```python
from build123d import *
from build123d.topology import SkipClean

# Parameters (mm, degrees)
LUG_DEPTH                         = 19
LUG_PIN_HOLE_A_SKETCH_R           = 3
LUG_PIN_HOLE_A_6_DEPTH            = 19
LUG_PIN_HOLE_B_SKETCH_R           = 3
LUG_PIN_HOLE_B_6_DEPTH            = 19
LUG_PATTERN_3X120_COUNT           = 3
LUG_CHAMFER_4MM_SIZE              = 4
BORE_START                        = -3.5
BORE_RECESS_SKETCH_R              = 10
BORE_RECESS_20_X3_5_DEPTH         = 3.5
CENTRE_BORE_SKETCH_R              = 10
CENTRE_BORE_20_X7_DEPTH           = 7
COUNTERBORE_SKETCH_R              = 13
COUNTERBORE_26_X2_5_DEPTH         = 2.5
RADIAL_SLOT_PROFILE_R             = 4.75
RADIAL_SLOT_DEPTH                 = 5
FLANGE_HOLE_SKETCH_R              = 2.75
FLANGE_HOLE_5_5_DEPTH             = 50.979995998
SLOT_AND_HOLE_PATTERN_3X120_COUNT = 3


with BuildPart() as part:
    # Base Flange Profile → Base Flange Ø62 (revolve)
    with BuildSketch(Plane.XY):
        with BuildLine():
            Line((-31, 4), (-31, -4))
            Line((-31, -4), (-17, -4))
            Line((-17, -4), (-17, -7))
            Line((-17, -7), (-19, -7))
            ThreePointArc((-19, -7), (-19.707106781, -7.292893219), (-20, -8))
            Line((-20, -8), (-20, -9))
            Line((-20, -9), (0, -9))
            Line((0, -9), (0, 4))
            Line((0, 4), (-31, 4))
        make_face()
    revolve(axis=Axis((0, 39.539668131, 0), (0, -1, 0)))

    # Lug Profile → Lug (add)
    with SkipClean():  # the faces are left unmerged after this step: merging them gives an invalid solid
        with BuildSketch(Plane(origin=(0, 4, 0), x_dir=(1, 0, 0), z_dir=(0, 1, 0))):
            with BuildLine():
                Line((5, 30.594117082), (5, 8.660254038))
                ThreePointArc((5, 8.660254038), (8.660254038, 5), (10, 0))
                Line((10, 0), (28.995282599, -10.966931522))
                ThreePointArc((28.995282599, -10.966931522), (29.806622049, -8.518525814), (30.411611519, -6.011146713))
                Line((30.411611519, -6.011146713), (10, 5.773502692))
                Line((10, 5.773502692), (10, 29.342801502))
                ThreePointArc((10, 29.342801502), (7.526051267, 30.072554802), (5, 30.594117082))
            make_face()
        lug = extrude(amount=LUG_DEPTH)

    # Lug Pin Hole A Sketch → Lug Pin Hole A Ø6 (cut)
    with SkipClean():  # the faces are left unmerged after this step: merging them gives an invalid solid
        with BuildSketch(Plane.ZY.offset(-5)):
            with Locations((-25.594117082, 15)):
                Circle(LUG_PIN_HOLE_A_SKETCH_R)
        lug_pin_hole_a_6 = extrude(amount=-LUG_PIN_HOLE_A_6_DEPTH, mode=Mode.SUBTRACT)

    # Lug Pin Hole B Sketch → Lug Pin Hole B Ø6 (cut)
    with SkipClean():  # the faces are left unmerged after this step: merging them gives an invalid solid
        with BuildSketch(Plane(origin=(2.5, 0, -4.330127019), x_dir=(0.8660254037844399, 0, 0.4999999999999978), z_dir=(-0.4999999999999978, 0, 0.8660254037844399))):
            with Locations((25.594117082, 15)):
                Circle(LUG_PIN_HOLE_B_SKETCH_R)
        lug_pin_hole_b_6 = extrude(amount=-LUG_PIN_HOLE_B_6_DEPTH, mode=Mode.SUBTRACT)

    # Lug Pattern 3x120°: Lug, Lug Pin Hole A Ø6, Lug Pin Hole B Ø6 ×3 about axis
    with SkipClean():  # the faces are left unmerged after this step: merging them gives an invalid solid
        lug_pattern_3x120_axis = Axis((0, 0, 0), (0, 1, 0))
        add([lug.rotate(lug_pattern_3x120_axis, i * 360 / LUG_PATTERN_3X120_COUNT) for i in range(1, LUG_PATTERN_3X120_COUNT)])
        add([lug_pin_hole_a_6.rotate(lug_pattern_3x120_axis, i * 360 / LUG_PATTERN_3X120_COUNT) for i in range(1, LUG_PATTERN_3X120_COUNT)], mode=Mode.SUBTRACT)
        add([lug_pin_hole_b_6.rotate(lug_pattern_3x120_axis, i * 360 / LUG_PATTERN_3X120_COUNT) for i in range(1, LUG_PATTERN_3X120_COUNT)], mode=Mode.SUBTRACT)

    # Lug Chamfer 4mm
    lug_chamfer_4mm_edges = [part.edges().sort_by_distance(p)[0] for p in [
        (29.806622049, 23, 8.518525814),
        (7.526051267, 23, -30.072554802),
        (-7.526051267, 23, -30.072554802),
        (-29.806622049, 23, 8.518525814),
        (-22.280570782, 23, 21.554028988),
        (22.280570782, 23, 21.554028988),
    ]]
    chamfer(lug_chamfer_4mm_edges, length=LUG_CHAMFER_4MM_SIZE)

    # Bore Recess Sketch → Bore Recess Ø20 x3.5 (cut)
    with BuildSketch(Plane(origin=(0, 4, 0), x_dir=(1, 0, 0), z_dir=(0, 1, 0)).offset(BORE_START)):
        with Locations(Location((0, 0, 0), (0, 0, 180))):
            Circle(BORE_RECESS_SKETCH_R)
    extrude(amount=BORE_RECESS_20_X3_5_DEPTH, mode=Mode.SUBTRACT)

    # Centre Bore Sketch → Centre Bore Ø20 x7 (cut)
    with BuildSketch(Plane.XZ.offset(9)):
        with Locations(Location((0, 0, 0), (0, 0, 180))):
            Circle(CENTRE_BORE_SKETCH_R)
    extrude(amount=-CENTRE_BORE_20_X7_DEPTH, mode=Mode.SUBTRACT)

    # Counterbore Sketch → Counterbore Ø26 x2.5 (cut)
    with BuildSketch(Plane.XZ.offset(2)):
        Circle(COUNTERBORE_SKETCH_R)
    extrude(amount=-COUNTERBORE_26_X2_5_DEPTH, mode=Mode.SUBTRACT)

    # Radial Slot Profile → Radial Slot (cut)
    with BuildSketch(Plane(origin=(0, 4, 0), x_dir=(1, 0, 0), z_dir=(0, 1, 0))):
        with Locations(Location((-6.470476128, -24.148145657, 0), (0, 0, 180))):
            Circle(RADIAL_SLOT_PROFILE_R)
    radial_slot = extrude(amount=-RADIAL_SLOT_DEPTH, mode=Mode.SUBTRACT)

    # Flange Hole Sketch → Flange Hole Ø5.5 (cut, through all)
    with BuildSketch(Plane(origin=(0, -1, 0), x_dir=(1, 0, 0), z_dir=(0, 1, 0))):
        with Locations(Location((-6.470476128, -24.148145657, 0), (0, 0, 180))):
            Circle(FLANGE_HOLE_SKETCH_R)
    flange_hole_5_5 = extrude(amount=-FLANGE_HOLE_5_5_DEPTH, mode=Mode.SUBTRACT)

    # Slot and Hole Pattern 3x120°: Radial Slot, Flange Hole Ø5.5 ×3 about axis
    slot_and_hole_pattern_3x120_axis = Axis((0, 0, 0), (0, 1, 0))
    add([radial_slot.rotate(slot_and_hole_pattern_3x120_axis, i * 360 / SLOT_AND_HOLE_PATTERN_3X120_COUNT) for i in range(1, SLOT_AND_HOLE_PATTERN_3X120_COUNT)], mode=Mode.SUBTRACT)
    add([flange_hole_5_5.rotate(slot_and_hole_pattern_3x120_axis, i * 360 / SLOT_AND_HOLE_PATTERN_3X120_COUNT) for i in range(1, SLOT_AND_HOLE_PATTERN_3X120_COUNT)], mode=Mode.SUBTRACT)


solid = part.part
```
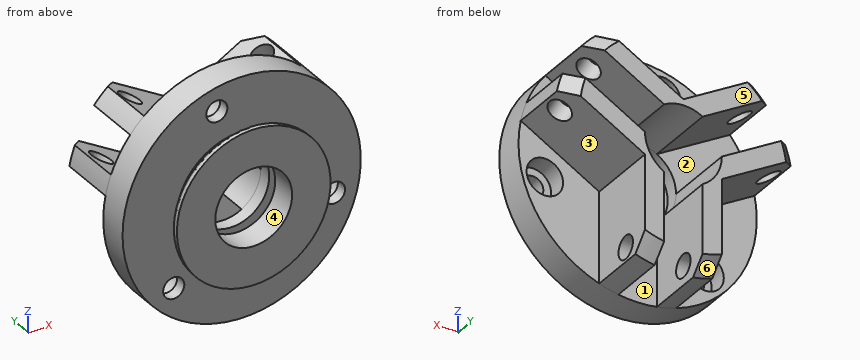
Model file for the job. Use its own axes, mm. Face numbers are marked on the shaded views. A direction names the side the tool comes from. Coordinates: 2 decimals unless noted, no trailing zeros. Loops run counter-clockwise (first coordinate to the right, second up) from the corner with the lowest first, then second, coordinate; pieces in that order, holes last. Notation, with made-up numbers: (70.5, 53.25) - (81.5, 53.25) arc R17 cw to (81.5, 83.25) - close; hole circle Ø6 at (8, 34). An arc over 180 degrees is marked (long way). Write item = value, one per line. Start each with the question number.
Item 1: Saw through at A-A, the plane y = 2. List the corners of the cut face in (x, z), then the cut area to 3 significant figures.
Item 2: Wall check: probe 1 along Y at (x, z) = (-3, -12.5); probe 2 along Z at (x, y) = (0.5, 2.5); probe 3 along Z at (x, y) = (-9, 1). Give the ranges that are in metal, low to high. Write a range as [from, to].
Item 3: Saw through at C-C, the plane y = 15. State how many separate pieces and enclosed holes the cut face has, then the cut area to 3 significant figures.
Item 4: Saw through at B-B, the plane y = -5. List the corners of the cut face in (x, z).
Item 5: Pull direction Z, two halves, no side cores. Call the marked faces 4, 5 and 6: +Z half, -Z half, draft (parallel to the pull), parting line (faces both ways), or undercut.
Item 6: Drop flat-ended pins along their axis: pin 1 Ø7 at (y, z) = (15, -25.59) entering from -X; pin 2 Ø1 at (y, z) = (-5.5, -5.5) entering from +X; pin 3 Ø3 at (x, y) = (15, 7) entering from -Z. Give the stop position or say it passes through.
Item 7: 3-axis set-ups, long thin cutter, end or side, ignore diameter. For the marked faces 1, 2 and 3: which of +Z, -Z, +X, -X, +Y, -Y reach the whole face in a straight line?
Answers:
q1.outline = circle Ø62 at (0, 0); hole circle Ø9.5 at (-17.68, -17.68); hole circle Ø9.5 at (-6.47, 24.15); hole circle Ø20 at (0, 0); hole circle Ø9.5 at (24.15, -6.47)
q1.area = 2,490 mm2
q2.probe_1 = [-9, -2], [0.5, 4]
q2.probe_2 = [-31, -9.99], [9.99, 31]
q2.probe_3 = [-29.66, -4.36], [4.36, 20.13], [28.17, 29.66]
q3.separate_pieces = 9
q3.enclosed_holes = 0
q3.area = 521 mm2
q4.outline = circle Ø34 at (0, 0); hole circle Ø20 at (0, 0)
q5.face_4 = undercut
q5.face_5 = draft
q5.face_6 = -Z half
q6.pin_1 = -10
q6.pin_2 = 16.25
q6.pin_3 = -3.75
q7.face_1 = -Z, +Y
q7.face_2 = +Y
q7.face_3 = -Z, +X, +Y
